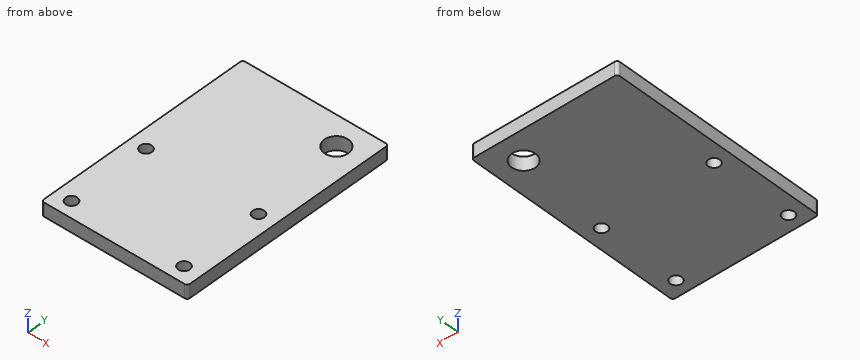
```python
from build123d import *

# Parameters (mm, degrees)
SKETCH_1_W                  = 107
SKETCH_1_H                  = 162
EXTRUDE_1_DEPTH             = 5
HOLE_WIZARD_M20_1_D         = 17.5
FILLET_1_R                  = 2
HOLE_WIZARD_M10_1_D         = 8.5
PATTERN_LINEAR_1_COUNT      = 2
PATTERN_LINEAR_1_PITCH      = 82.5
PATTERN_LINEAR_1_COUNT_DIR2 = 2
PATTERN_LINEAR_1_PITCH_DIR2 = 60


with BuildPart() as part:
    # 草图1 → 凸台-拉伸1 (new, symmetric)
    with BuildSketch(Plane.XY):
        Rectangle(SKETCH_1_W, SKETCH_1_H)
    extrude(amount=EXTRUDE_1_DEPTH, both=True)

    # M20 螺纹孔1 (through all)
    with Locations(Plane.XY.offset(5)):
        with Locations((33.5, 61)):
            Hole(HOLE_WIZARD_M20_1_D / 2)

    # 圆角1
    fillet_1_edges = [part.edges().sort_by_distance(p)[0] for p in [
        (53.5, -81, 0),
        (-53.5, -81, 0),
        (-53.5, 81, 0),
        (53.5, 81, 0),
    ]]
    fillet(fillet_1_edges, radius=FILLET_1_R)

    # M10 螺纹孔1 (through all)
    with Locations(Plane.XY.offset(5)):
        with Locations((-41.5, -70)):
            hole_wizard_m10_1 = Hole(HOLE_WIZARD_M10_1_D / 2)

    # 阵列(线性)1: Hole Wizard M10 _1 2 × 2
    with Locations(*[(i * PATTERN_LINEAR_1_PITCH, j * PATTERN_LINEAR_1_PITCH_DIR2, 0) for i in range(PATTERN_LINEAR_1_COUNT) for j in range(PATTERN_LINEAR_1_COUNT_DIR2) if (i, j) != (0, 0)]):
        add(hole_wizard_m10_1, mode=Mode.SUBTRACT)


solid = part.part
```
For this review, take the finished solid that the model builds, in its own axes (mm). Round coordinates to 2 decimals unless told otherwise and drop trailing zeros. Loops run counter-clockwise (first coordinate to the right, second up) from the corner with the lowest first, then second, coordinate; pieces in that order, holes last.
Q1. Insertion check: pin 1 Ø5 at (x, y) = (-41.5, -10) entering from -Z; pin 2 Ø23 at (x, y) = (33.5, 61) entering from -Z. Each pin has a flat end and moves straight along its axis. Give the tip position at first contact, or say it passes through.
Result sheet:
pin 1: passes through
pin 2: stops at z = -5
Q2. Add section D-D on z = 1.5. Write out the cut boundary in (x, y), plus the area to 3 significant figures.
Result sheet:
outline: (-53.5, -79) arc R2 ccw to (-51.5, -81) - (51.5, -81) arc R2 ccw to (53.5, -79) - (53.5, 79) arc R2 ccw to (51.5, 81) - (-51.5, 81) arc R2 ccw to (-53.5, 79) - close; hole circle Ø8.5 at (-41.5, -70); hole circle Ø8.5 at (-41.5, -10); hole circle Ø17.5 at (33.5, 61); hole circle Ø8.5 at (41, -70); hole circle Ø8.5 at (41, -10)
area: 16,900 mm2
Q3. Add section A-A on x = -39.5. Write out the cut boundary in (y, z), plus the area to 3 significant figures.
Result sheet:
outline: (-81, -5) - (-73.75, -5) - (-73.75, 5) - (-81, 5) - close; (-66.25, -5) - (-13.75, -5) - (-13.75, 5) - (-66.25, 5) - close; (-6.25, -5) - (81, -5) - (81, 5) - (-6.25, 5) - close
area: 1,470 mm2
Q4. Add section B-B on y = -68. Write out the cut boundary in (x, z), plus the area to 3 significant figures.
Result sheet:
outline: (-53.5, -5) - (-45.25, -5) - (-45.25, 5) - (-53.5, 5) - close; (-37.75, -5) - (37.25, -5) - (37.25, 5) - (-37.75, 5) - close; (44.75, -5) - (53.5, -5) - (53.5, 5) - (44.75, 5) - close
area: 920 mm2
Q5. Add section C-C on x = 33.5. Write out the cut boundary in (y, z), plus the area to 4 significant figures.
Result sheet:
outline: (-81, -5) - (52.25, -5) - (52.25, 5) - (-81, 5) - close; (69.75, -5) - (81, -5) - (81, 5) - (69.75, 5) - close
area: 1,445 mm2
Q6. To check wall thickness, follow line 1 along Y through (x, z) = (-41.5, -1.25); line 2 along Y through (x, z) = (41, -2); line 3 along Y through (x, z) = (29.5, -4). State the ranges of each line that lie inside material, in increasing order.
Result sheet:
line 1: y = -81 to -74.25, -65.75 to -14.25, -5.75 to 81
line 2: y = -81 to -74.25, -65.75 to -14.25, -5.75 to 56.49, 65.51 to 81
line 3: y = -81 to 53.22, 68.78 to 81
